Check sheet for the modelled part. Datum: model origin and axes. Units: mm. Face numbers are marked on the shaded views. Coordinates: 2 decimals unless noted, no trailing zeros. Loops run counter-clockwise (first coordinate to the right, second up) from the corner with the lowest first, then second, coordinate; pieces in that order, holes last.
```python
from build123d import *

# Parameters (mm, degrees)
SKETCH1_W           = 18.701399688
SKETCH1_H           = 9.037325038
SKETCH1_R           = 1.1
BOSS_EXTRUDE1_DEPTH = 2
SKETCH2_W           = 18.701399688
SKETCH2_H           = 15
SKETCH2_R           = 3.439163943
BOSS_EXTRUDE2_DEPTH = 2


with BuildPart() as part:
    # Sketch1 → Boss-Extrude1 (new body)
    with BuildSketch(Plane(origin=(0, 0, 0), x_dir=(1, 0, 0), z_dir=(0, 1, 0))):
        Rectangle(SKETCH1_W, SKETCH1_H)
        with Locations(Location((-6.196734059, 0, 0), (0, 0, 270))):
            Circle(SKETCH1_R, mode=Mode.SUBTRACT)
        with Locations(Location((6.803265941, 0, 0), (0, 0, 270))):
            Circle(SKETCH1_R, mode=Mode.SUBTRACT)
    extrude(amount=BOSS_EXTRUDE1_DEPTH)

    # Sketch2 → Boss-Extrude2 (add)
    with BuildSketch(Plane.XY.offset(4.518662519)):
        with Locations((0, 7.5)):
            Rectangle(SKETCH2_W, SKETCH2_H)
        with Locations((0, 9.421314685)):
            Circle(SKETCH2_R, mode=Mode.SUBTRACT)
    extrude(amount=BOSS_EXTRUDE2_DEPTH)


solid = part.part
```
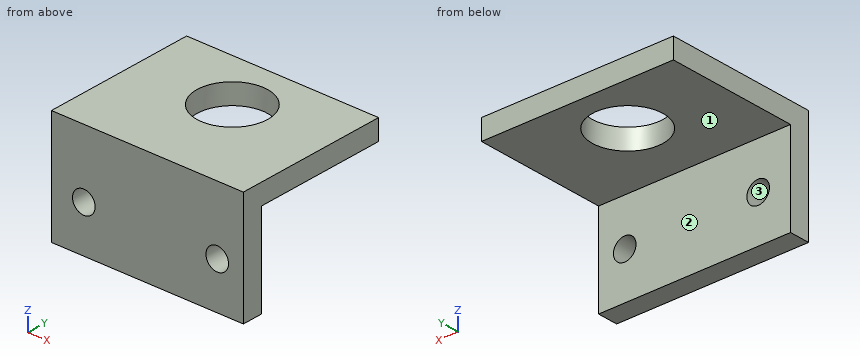
1) Mould release check, pull along Z, two halves, no side actions. Record for the marked faces 1, 2 and 3: +Z half, -Z half, draft (parallel to the pull), parting line (faces both ways), or undercut.
Answer sheet:
face 1: -Z half
face 2: draft
face 3: undercut
2) Section check D-D on y = 1.75. Enter the section's corners in (x, z).
Answer sheet:
outline: (-9.35, -4.52) - (9.35, -4.52) - (9.35, 6.52) - (-9.35, 6.52) - close; hole circle Ø2.2 at (-6.2, 0); hole circle Ø2.2 at (6.8, 0)
3) Depth check by flat-ended pin: pin 1 (5 mm diameter, centred on x = 2, y = 8.5, fed in from -Z); pin 2 (2.5 mm diameter, centred on x = 3, z = 1, fed in from +Y). Enter the tip coordinate at first touch or a pass-through.
Answer sheet:
pin 1: stops at z = 4.52
pin 2: stops at y = 2
4) Scan lines: line 1 (X direction, y = 1.5, z = 0); line 2 (Z direction, x = -3.75, y = 8.5); line 3 (Y direction, x = -0.5, z = 2). Record each from-to range of solid material in increasing order.
Answer sheet:
line 1: x = -9.35 to -7.3, -5.1 to 5.7, 7.9 to 9.35
line 2: z = 4.52 to 6.52
line 3: y = 0 to 2
5) Section check C-C on y = 10.5. Enter the section's corners in (x, z), plus the area to 3 significant figures.
Answer sheet:
outline: (-9.35, 4.52) - (-3.27, 4.52) - (-3.27, 6.52) - (-9.35, 6.52) - close; (3.27, 4.52) - (9.35, 4.52) - (9.35, 6.52) - (3.27, 6.52) - close
area: 24.3 mm2
6) Section check A-A on x = 0. Enter the section's corners in (y, z).
Answer sheet:
outline: (0, -4.52) - (2, -4.52) - (2, 4.52) - (5.98, 4.52) - (5.98, 6.52) - (0, 6.52) - close; (12.86, 4.52) - (15, 4.52) - (15, 6.52) - (12.86, 6.52) - close
7) Section check B-B on z = 0. Enter the section's corners in (x, y).
Answer sheet:
outline: (-9.35, 0) - (-7.3, 0) - (-7.3, 2) - (-9.35, 2) - close; (-5.1, 0) - (5.7, 0) - (5.7, 2) - (-5.1, 2) - close; (7.9, 0) - (9.35, 0) - (9.35, 2) - (7.9, 2) - close
